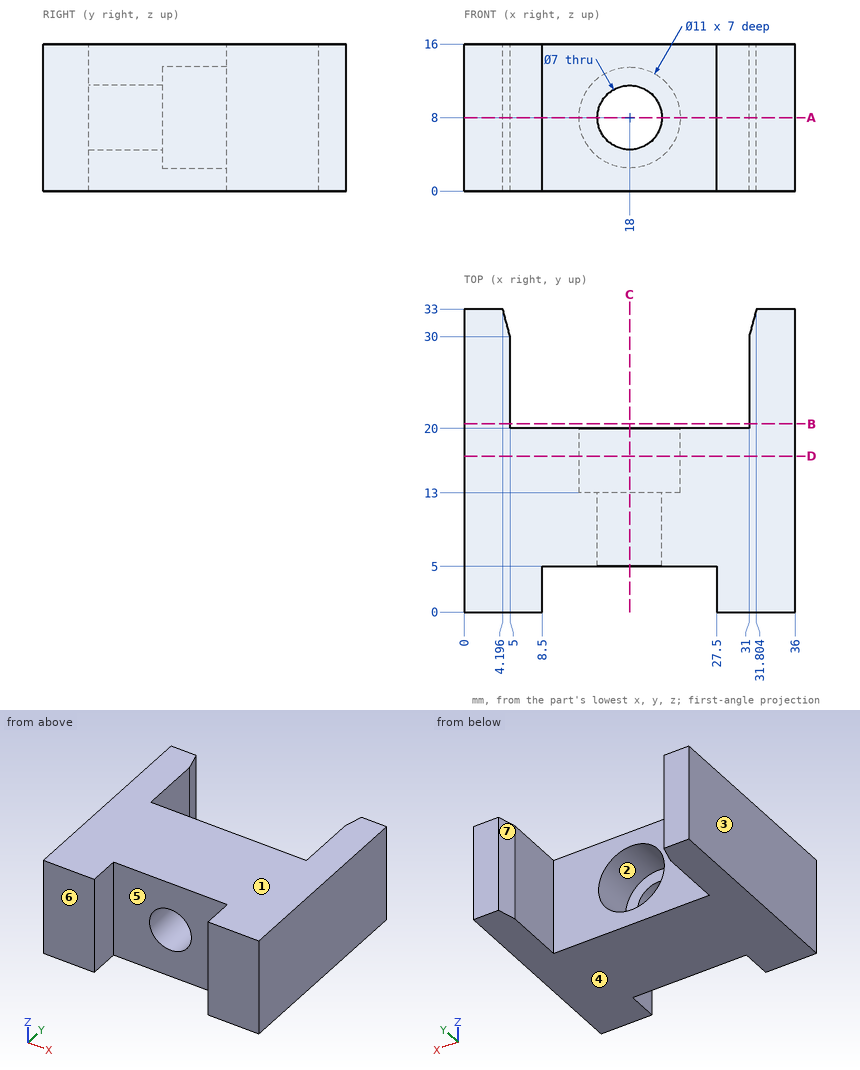
Geometry check sheet. Reference: drawing and pictorial views, mm from the part's lowest x, y, z. A direction names the side the tool comes from. Coordinates: 2 decimals unless noted, no trailing zeros. Loops run counter-clockwise (first coordinate to the right, second up) from the corner with the lowest first, then second, coordinate; pieces in that order, holes last. Notation, with made-up numbers: (40.25, -1.75) - (69.25, -1.75) arc R22 cw to (69.25, 29.25) - close; hole circle Ø11 at (65, -38). An arc over 180 degrees is marked (long way). Return JSON: item names as keys, results as strings.
1. Section check D-D, the plane y = 17. Record the boundary of the cut face in (x, z).
Established:
{"outline": "(0, 0) - (36, 0) - (36, 16) - (0, 16) - close; hole circle Ø11 at (18, 8)"}
2. Tool access check on the marked faces 5, 6 and 7. Record the directions out of +Z, -Z, +X, -X, +Y, -Y that give a thin tool (end or side, any length) a straight path to the whole face; none if there is none.
Established:
{"face 5": "+Z, -Z, -Y", "face 6": "+Z, -Z, +X, -X, -Y", "face 7": "+Z, -Z, +Y"}
3. Section check A-A, the plane z = 8. Record the boundary of the cut face in (x, y).
Established:
{"outline": "(0, 0) - (8.5, 0) - (8.5, 5) - (14.5, 5) - (14.5, 13) - (12.5, 13) - (12.5, 20) - (5, 20) - (5, 30) - (4.2, 33) - (0, 33) - close; (21.5, 5) - (27.5, 5) - (27.5, 0) - (36, 0) - (36, 33) - (31.8, 33) - (31, 30) - (31, 20) - (23.5, 20) - (23.5, 13) - (21.5, 13) - close"}
4. Go/stop test with flat-tipped pins: pin 1 (5.5 mm diameter, centred on x = 18.5, z = 9, fed in from +Y); pin 2 (1 mm diameter, centred on x = 15, z = 2.5, fed in from -Y); pin 3 (4 mm diameter, centred on x = 13, z = 9.5, fed in from +Y). Record where each tip stops, or that it passes through.
Established:
{"pin 1": "stops at y = 13", "pin 2": "stops at y = 5", "pin 3": "stops at y = 20"}
5. Section check C-C, the plane x = 18. Record the boundary of the cut face in (y, z).
Established:
{"outline": "(5, 0) - (20, 0) - (20, 2.5) - (13, 2.5) - (13, 4.5) - (5, 4.5) - close; (5, 11.5) - (13, 11.5) - (13, 13.5) - (20, 13.5) - (20, 16) - (5, 16) - close"}
6. Mould release check, pull along Z, two halves, no side actions. Record for the marked faces 1, 2, 3 and 4: +Z half, -Z half, draft (parallel to the pull), parting line (faces both ways), or undercut.
Established:
{"face 1": "+Z half", "face 2": "undercut", "face 3": "draft", "face 4": "-Z half"}
7. Thickness scan on L1, parallel to X at y = 28.5, z = 5; L2, parallel to X at y = 10, z = 8; L3, parallel to Y at x = 30.5, z = 7. Record the ranges inside material, lowest first.
Established:
{"L1": "x = 0 to 5, 31 to 36", "L2": "x = 0 to 14.5, 21.5 to 36", "L3": "y = 0 to 20"}
8. Section check B-B, the plane y = 20.5. Record the boundary of the cut face in (x, z).
Established:
{"outline": "(0, 0) - (5, 0) - (5, 16) - (0, 16) - close; (31, 0) - (36, 0) - (36, 16) - (31, 16) - close"}
